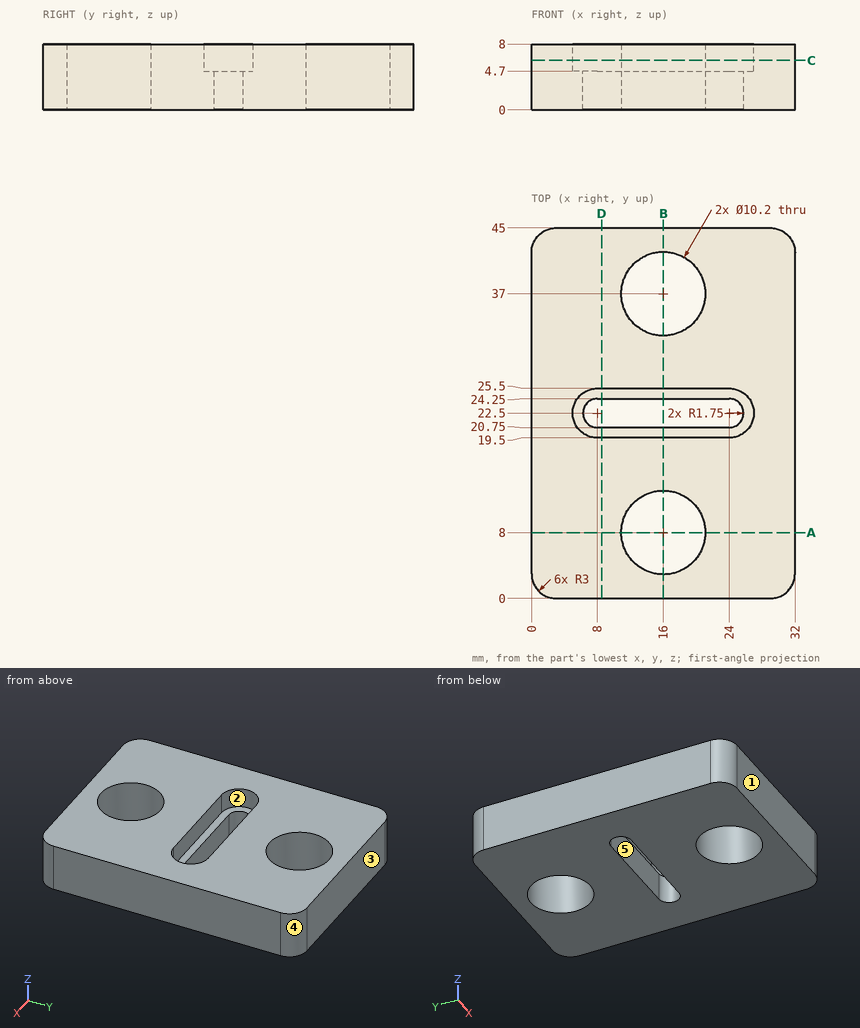
Study the drawing (mm; zero at the part's minimum x, y, z) and answer. A direction names the side the tool comes from. Give positions to 0.01 mm unless a question says otherwise; leave off trailing zeros. Loops run counter-clockwise (first coordinate to the right, second up) from the corner with the lowest first, then second, coordinate; pieces in that order, holes last. Notation, with made-up numbers: (83, -23.5) - (139, -23.5) arc R10 ccw to (139, -18.5) - close; hole circle Ø3 at (38, 7). An arc over 180 degrees is marked (long way). Return JSON: item names as keys, results as strings. Group by question number.
1. Given pin 1 Ø6 at (x, y) = (16.5, 38.5) entering from +Z; pin 2 Ø5 at (x, y) = (14, 22.5) entering from +Z, each flat-ended and moving along its own axis, determine where each tip first touches the part or whether it passes through.
2. Find section A-A (y = 8). Write down the section's boundary in (x, z).
3. Find section B-B (x = 16). Write down the section's boundary in (y, z).
4. Find section D-D (x = 8.5). Write down the section's boundary in (y, z), then the cut area to 3 significant figures.
5. Which of the six approach directions +Z, -Z, +X, -X, +Y, -Y give full straight-line access (tool end or side, diameter ignored) to the marked faces 4 and 5?
6. Straight lines are drawn through the part: line 1 (Y direction, x = 16, z = 3.5); line 2 (Y direction, x = 16, z = 6.75); line 3 (Y direction, x = 10.5, z = 3). For each, find the intervals that lie inside material, in ascending order. Write a range as [from, to].
7. Find section C-C (z = 6). Write down the section's boundary in (x, y), then the cut area to 3 significant figures.
8. Determine the mould class of the marked faces 1, 2 and 3 for opening direction Y: pulls with the +Y half, pulls with the -Y half, needs draft (parallel to the pull), parting line crosses it, or undercut.
Verdict:
{
 "1": {"pin 1": "passes through", "pin 2": "stops at z = 4.7"},
 "2": {"outline": "(0, 0) - (10.9, 0) - (10.9, 8) - (0, 8) - close; (21.1, 0) - (32, 0) - (32, 8) - (21.1, 8) - close"},
 "3": {"outline": "(0, 0) - (2.9, 0) - (2.9, 8) - (0, 8) - close; (13.1, 0) - (20.75, 0) - (20.75, 4.7) - (19.5, 4.7) - (19.5, 8) - (13.1, 8) - close; (24.25, 0) - (31.9, 0) - (31.9, 8) - (25.5, 8) - (25.5, 4.7) - (24.25, 4.7) - close; (42.1, 0) - (45, 0) - (45, 8) - (42.1, 8) - close"},
 "4": {"outline": "(0, 0) - (20.75, 0) - (20.75, 4.7) - (19.5, 4.7) - (19.5, 8) - (0, 8) - close; (24.25, 0) - (45, 0) - (45, 8) - (25.5, 8) - (25.5, 4.7) - (24.25, 4.7) - close", "area": "324 mm^2"},
 "5": {"face 4": "+Z, -Z, +X, +Y", "face 5": "+Z, -Z"},
 "6": {"line 1": "y = [0, 2.9], [13.1, 20.75], [24.25, 31.9], [42.1, 45]", "line 2": "y = [0, 2.9], [13.1, 19.5], [25.5, 31.9], [42.1, 45]", "line 3": "y = [0, 20.75], [24.25, 45]"},
 "7": {"outline": "(0, 3) arc R3 ccw to (3, 0) - (29, 0) arc R3 ccw to (32, 3) - (32, 42) arc R3 ccw to (29, 45) - (3, 45) arc R3 ccw to (0, 42) - close; hole (8, 19.5) - (24, 19.5) arc R3 ccw to (24, 25.5) - (8, 25.5) arc R3 ccw to start; hole circle Ø10.2 at (16, 8); hole circle Ø10.2 at (16, 37)", "area": "1,140 mm^2"},
 "8": {"face 1": "pulls with the -Y half", "face 2": "undercut", "face 3": "pulls with the +Y half"}
}
